```python
from build123d import *

# Parameters (mm, degrees)
SKETCH_6_R             = 17.5
EXTRUDE_3_DEPTH        = 6
SKETCH_7_R             = 10
CUT_EXTRUDE_1_DEPTH    = 10
SKETCH_8_R             = 3.1
CUT_EXTRUDE_2_DEPTH    = 10
CUT_EXTRUDE_3_DEPTH    = 83.598426135
CHAMFER_1_SIZE         = 1
HOLE_WIZARD_M3_1_D     = 2.5
HOLE_WIZARD_M3_1_DEPTH = 8.5
HOLE_WIZARD_M3_1_TIP   = 0.751075774


with BuildPart() as part:
    # 草图6 → 凸台-拉伸3 (new body)
    with BuildSketch(Plane.XY):
        with Locations((42.5, 0)):
            Circle(SKETCH_6_R)
        with BuildLine():
            Line((-42.5, 10), (42.5, 10))
            ThreePointArc((42.5, 10), (52.5, 0), (42.5, -10))
            Line((42.5, -10), (-42.5, -10))
            ThreePointArc((-42.5, -10), (-52.5, 0), (-42.5, 10))
        make_face()
    extrude(amount=EXTRUDE_3_DEPTH)

    # 草图7 → 切除-拉伸1 (cut)
    with BuildSketch(Plane(origin=(0, 0, 0), x_dir=(-1, 0, 0), z_dir=(0, 0, -1))):
        with Locations((-42.5, 0)):
            Circle(SKETCH_7_R)
    extrude(amount=-CUT_EXTRUDE_1_DEPTH, mode=Mode.SUBTRACT)

    # 草图8 → 切除-拉伸2 (cut)
    with BuildSketch(Plane(origin=(0, 0, 0), x_dir=(-1, 0, 0), z_dir=(0, 0, -1))):
        with Locations((42.5, 0)):
            Circle(SKETCH_8_R)
    extrude(amount=-CUT_EXTRUDE_2_DEPTH, mode=Mode.SUBTRACT)

    # 草图9 → 切除-拉伸3 (cut, through all)
    with BuildSketch(Plane(origin=(28, 0, 0), x_dir=(0, 0, -1), z_dir=(1, 0, 0))):
        Polygon((-4, -10), (-6, 0), (-6, -10), align=None)
        Polygon((-2, -10), (0, 0), (0, -10), align=None)
    extrude(amount=-CUT_EXTRUDE_3_DEPTH, mode=Mode.SUBTRACT)

    # 倒角1
    chamfer_1_edges = [part.edges().sort_by_distance(p)[0] for p in [
        (60, 0, 6),
        (52.5, 0, 6),
        (52.5, 0, 0),
        (60, 0, 0),
    ]]
    chamfer(chamfer_1_edges, length=CHAMFER_1_SIZE)

    # M3 螺纹孔1
    with Locations(Plane(origin=(0, 0, 0), x_dir=(-1, 0, 0), z_dir=(0, 0, -1))):
        with Locations((-14.611830465, 2.5)):
            Hole(HOLE_WIZARD_M3_1_D / 2, depth=HOLE_WIZARD_M3_1_DEPTH)
            with Locations((0, 0, -(HOLE_WIZARD_M3_1_DEPTH + HOLE_WIZARD_M3_1_TIP / 2))):  # 118° drill point
                Cone(0, HOLE_WIZARD_M3_1_D / 2, HOLE_WIZARD_M3_1_TIP, mode=Mode.SUBTRACT)


solid = part.part
```
Here's how the part is built. I have some questions about the finished solid (model axes, mm). A direction names the side the tool comes from. Give positions to 0.01 mm unless a question says otherwise; leave off trailing zeros. Loops run counter-clockwise (first coordinate to the right, second up) from the corner with the lowest first, then second, coordinate; pieces in that order, holes last. Notation, with made-up numbers: M -40,-7 L 14,-7 A28 cw 14,18 Z; hole C -7.75,-23 d2. An arc over 180 degrees is marked long. Put each result on its own line as item: value. Start each with the question number.
(1) Will these pins go through, and if not, where does the flat tip stop? pin 1 Ø3 at (y, z) = (7.5, 3) entering from -X; pin 2 Ø1 at (x, y) = (-19, -3.5) entering from -Z; pin 3 Ø0.6 at (y, z) = (-5.5, 0.5) entering from -X; pin 4 Ø5.5 at (x, y) = (-42.5, 0) entering from -Z.
(2) I want a section at A-A on x = 42.5. Please give me the cut outline in (y, z), then the cut area to 3 significant figures.
(3) I need wall thicknesses on line 1 along Y through (x, z) = (42.5, 3.35); line 2 along X through (y, z) = (5, 1.25); line 3 along X through (y, z) = (-4.5, 2.5). Which ranges of each line are inside material? Lowest first, please. Write a range as [from, to].
(4) I want a section at B-B on z = 3. Please give me the cut outline in (x, y).
(5) For faces 4 (the flat face through (28, -7, 1)), 5 (the flat face through (-12, -5, 5)), 6 (the cylindrical face through (52.49, 0.44, 2.97)), which set-ups out of +Z, -Z, +X, -X, +Y, -Y let a thin tool reach every point of the face, with its end or its side?
(6) If we mould it in two halves opening along X, with no side actions, what happens to faces 1 (the cylindrical face through (13.363, 2.555, 3.042)), 2 (the conical face through (59.15, -0.59, 5.84)), 3 (the flat face through (-7, 10, 3))? For each: +X half, -X half, draft (parallel to the pull), parting line (faces both ways), or undercut.
(7) I want a section at C-C on x = -25.5. Please give me the cut outline in (y, z), then the cut area to 3 significant figures.
Answer block:
1. pin 1: x = -50.5
1. pin 2: z = 0.6
1. pin 3: x = 28
1. pin 4: through
2. outline: M -17.5,1 L -16.5,0 L -11,0 L -10,1 L -10,5 L -11,6 L -16.5,6 L -17.5,5 Z; M 10,1 L 11,0 L 16.5,0 L 17.5,1 L 17.5,5 L 16.5,6 L 11,6 L 10,5 Z
2. area: 86.0 mm^2
3. line 1: [-17.5, -10], [10, 17.5]
3. line 2: [-51.16, 33.84], [51.16, 59.27]
3. line 3: [-51.43, 33.57], [51.43, 59.41]
4. outline: M -42.5,-10 L 28.14,-10 A17.5 ccw long 28.14,10 L -42.5,10 A10 ccw Z; hole C -42.5,0 d6.2; hole C 14.61,2.5 d2.5; hole C 42.5,0 d20
5. face 4: -Z, -X, -Y
5. face 5: +Z, -X, -Y
5. face 6: +Z, -Z
6. face 1: undercut
6. face 2: parting line
6. face 3: draft
7. outline: M -10,2 L 0,0 L 10,0 L 10,6 L 0,6 L -10,4 Z
7. area: 100 mm^2
